Can you work these out from the model? Positions are in its coordinate system, mm. A direction names the side the tool comes from. Give positions to 0.01 mm unless a question says otherwise; leave off trailing zeros. Write each loop counter-clockwise with the first axis right and the second up, starting at its lowest first coordinate (ties: lowest second). Pieces come first, ordered by that corner, then holes. Notation, with made-up numbers: (33.5, -8) - (51.5, -8) arc R35 ccw to (51.5, 25) - close; hole circle Ø5 at (59, -0.5). An arc over 180 degrees is marked (long way). Return JSON: item names as keys, results as strings. Group by question number.
from build123d import *


with BuildPart() as part:
    # Sketch1 → Revolve1 (revolve)
    with BuildSketch(Plane.XY):
        with BuildLine():
            Line((-15, 0), (-40, 0))
            Line((-40, 0), (-40, 1.432640688))
            Line((-40, 1.432640688), (-38.716216216, 1.914416082))
            ThreePointArc((-38.716216216, 1.914416082), (-34.5, 8), (-38.716216216, 14.085583918))
            Line((-38.716216216, 14.085583918), (-40, 14.567359312))
            Line((-40, 14.567359312), (-40, 16))
            Line((-40, 16), (-15, 16))
            Line((-15, 16), (-15, 21))
            Line((-15, 21), (-7.5, 21))
            Line((-7.5, 21), (-7.5, 24))
            Line((-7.5, 24), (0, 24))
            Line((0, 24), (0, -8))
            Line((0, -8), (-7.5, -8))
            Line((-7.5, -8), (-7.5, -5))
            Line((-7.5, -5), (-15, -5))
            Line((-15, -5), (-15, 0))
        make_face()
    revolve(axis=Axis((0, 24, 0), (0, -1, 0)))


solid = part.part
1) I need wall thicknesses on line 1 along Y through (x, z) = (15, 5); line 2 along Z through (x, y) = (13, 17); line 3 along Y through (x, z) = (18, 31). Which ranges of each line are inside material? Lowest first, please.
2) Imagine slicing it at D-D, the plane y = 19. Write out the boundary of the cut face in (x, z).
3) Imagine slicing it at C-C, the plane y = 7. Write out the boundary of the cut face in (x, z).
4) Imagine slicing it at A-A, the plane z = 0. Write out the boundary of the cut face in (x, y).
5) On a 3-axis mill with a long thin cutter (end or side, diameter ignored), from which of +Z, -Z, +X, -X, +Y, -Y can I reach the whole of each face in a straight line? I mean faces 1 (the face through (-4, -5, -7)), 2 (the face through (0, 24, 0)), 3 (the face through (7.493, 22.521, -0.33)). Say none if no direction works.
6) Imagine slicing it at B-B, the plane x = 0. Write out the boundary of the cut face in (y, z), and give its area (3 significant figures).
7) Will these pins go through, and if not, where does the flat tip stop? pin 1 Ø12 at (y, z) = (16.5, -21) entering from -X; pin 2 Ø10 at (x, z) = (-9.5, -8) entering from -Y; pin 3 Ø10 at (x, y) = (-8, 9) entering from +Z; pin 4 Ø4 at (x, y) = (31, 9.5) entering from -Z.
Resolved:
{
 "1": {"line 1": "0 to 16", "line 2": "-7.48 to 7.48", "line 3": "0 to 4.04, 11.96 to 16"},
 "2": {"outline": "circle Ø30 at (0, 0)"},
 "3": {"outline": "circle Ø69.15 at (0, 0)"},
 "4": {"outline": "(-40, 0) - (-15, 0) - (-15, -5) - (-7.5, -5) - (-7.5, -8) - (7.5, -8) - (7.5, -5) - (15, -5) - (15, 0) - (40, 0) - (40, 1.43) - (38.72, 1.91) arc R6.5 cw to (38.72, 14.09) - (40, 14.57) - (40, 16) - (15, 16) - (15, 21) - (7.5, 21) - (7.5, 24) - (-7.5, 24) - (-7.5, 21) - (-15, 21) - (-15, 16) - (-40, 16) - (-40, 14.57) - (-38.72, 14.09) arc R6.5 cw to (-38.72, 1.91) - (-40, 1.43) - close"},
 "5": {"face 1": "-Y", "face 2": "+Z, -Z, +X, -X, +Y", "face 3": "+Y"},
 "6": {"outline": "(-8, -7.5) - (-5, -7.5) - (-5, -15) - (0, -15) - (0, -40) - (1.43, -40) - (1.91, -38.72) arc R6.5 cw to (14.09, -38.72) - (14.57, -40) - (16, -40) - (16, -15) - (21, -15) - (21, -7.5) - (24, -7.5) - (24, 7.5) - (21, 7.5) - (21, 15) - (16, 15) - (16, 40) - (14.57, 40) - (14.09, 38.72) arc R6.5 cw to (1.91, 38.72) - (1.43, 40) - (0, 40) - (0, 15) - (-5, 15) - (-5, 7.5) - (-8, 7.5) - close", "area": "1,560 mm^2"},
 "7": {"pin 1": "x = -37.07", "pin 2": "y = -8", "pin 3": "z = 37.7", "pin 4": "z = -19.2"}
}
